from build123d import *

# Parameters (mm, degrees)
SKETCH1_W           = 20
SKETCH1_H           = 60
BOSS_EXTRUDE1_DEPTH = 15
CHAMFER1_SIZE       = 5
CUT_EXTRUDE1_DEPTH  = 36
CUT_EXTRUDE2_DEPTH  = 36
CUT_EXTRUDE3_DEPTH  = 6


with BuildPart() as part:
    # Sketch1 → Boss-Extrude1 (new body)
    with BuildSketch(Plane(origin=(0, 0, 0), x_dir=(1, 0, 0), z_dir=(0, 1, 0))):
        Rectangle(SKETCH1_W, SKETCH1_H)
    extrude(amount=BOSS_EXTRUDE1_DEPTH)

    # Chamfer1
    chamfer1_edges = [part.edges().sort_by_distance(p)[0] for p in [
        (-10, 15, 0),
    ]]
    chamfer(chamfer1_edges, length=CHAMFER1_SIZE)

    # Sketch2 → Cut-Extrude1 (cut, through all)
    with BuildSketch(Plane(origin=(0, 15, 0), x_dir=(1, 0, 0), z_dir=(0, 1, 0))):
        Polygon((10, -30), (9, -30), (10, -10), align=None)
    extrude(amount=-CUT_EXTRUDE1_DEPTH, mode=Mode.SUBTRACT)

    # Sketch3 → Cut-Extrude2 (cut, through all)
    with BuildSketch(Plane(origin=(0, 15, 0), x_dir=(1, 0, 0), z_dir=(0, 1, 0))):
        with BuildLine():
            Line((5, 21.75), (-1, 21.75))
            ThreePointArc((-1, 21.75), (-3.25, 24), (-1, 26.25))
            Line((-1, 26.25), (5, 26.25))
            ThreePointArc((5, 26.25), (7.25, 24), (5, 21.75))
        make_face()
    cut_extrude2 = extrude(amount=-CUT_EXTRUDE2_DEPTH, mode=Mode.SUBTRACT)

    # Sketch4 → Cut-Extrude3 (cut)
    with BuildSketch(Plane(origin=(0, 15, 0), x_dir=(1, 0, 0), z_dir=(0, 1, 0))):
        with BuildLine():
            Line((-1, 19.75), (5, 19.75))
            ThreePointArc((5, 19.75), (9.25, 24), (5, 28.25))
            Line((5, 28.25), (-1, 28.25))
            ThreePointArc((-1, 28.25), (-5.25, 24), (-1, 19.75))
        make_face()
    cut_extrude3 = extrude(amount=-CUT_EXTRUDE3_DEPTH, mode=Mode.SUBTRACT)

    # Mirror1: Cut-Extrude2, Cut-Extrude3 across plane
    add(cut_extrude2.mirror(Plane.XY), mode=Mode.SUBTRACT)
    add(cut_extrude3.mirror(Plane.XY), mode=Mode.SUBTRACT)


solid = part.part
Part model, mm, in its own coordinate system. A direction names the side the tool comes from. Coordinates: 2 decimals unless noted, no trailing zeros. Order: outer loops, then holes, each group sorted by start corner. A loop starts at its lowest first (then second) coordinate and runs counter-clockwise, first axis right, second up.
(1) Slice it at B-B, the plane x = 3.25. Write the cut outline in (y, z), and give its area (3 significant figures).
Check sheet entries:
outline: (0, -30) - (15, -30) - (15, -28.25) - (9, -28.25) - (9, -26.25) - (0, -26.25) - close; (0, -21.75) - (9, -21.75) - (9, -19.75) - (15, -19.75) - (15, 19.75) - (9, 19.75) - (9, 21.75) - (0, 21.75) - close; (0, 26.25) - (9, 26.25) - (9, 28.25) - (15, 28.25) - (15, 30) - (0, 30) - close
area: 717 mm2
(2) Pull direction X, two halves, no side cores. Call faces 1 (the face through (0, 7, -30)), 2 (the face through (-7, 13, 0)), 3 (the face through (2, 12, 19.75)): pulls with the +X half, pulls with the -X half, needs draft (parallel to the pull), parting line crosses it, or undercut.
Check sheet entries:
face 1: needs draft
face 2: pulls with the -X half
face 3: undercut
(3) Pin check, flat tip, straight feed: pin 1 Ø4 at (x, z) = (1, 22) entering from +Y. Stop position of the tip, or through.
Check sheet entries:
pin 1: stops at y = 9
(4) Slice it at A-A, the plane z = -24. Write the cut outline in (x, y).
Check sheet entries:
outline: (-10, 0) - (-3.25, 0) - (-3.25, 9) - (-5.25, 9) - (-5.25, 14.75) - (-10, 10) - close; (7.25, 0) - (10, 0) - (10, 15) - (9.25, 15) - (9.25, 9) - (7.25, 9) - close
(5) Slice it at C-C, the plane y = 12. Write the cut outline in (x, z), and give its area (3 significant figures).
Check sheet entries:
outline: (-8, -30) - (10, -30) - (10, 10) - (9, 30) - (-8, 30) - close; hole (-1, -28.25) - (5, -28.25) arc R4.25 ccw to (5, -19.75) - (-1, -19.75) arc R4.25 ccw to start; hole (-1, 19.75) - (5, 19.75) arc R4.25 ccw to (5, 28.25) - (-1, 28.25) arc R4.25 ccw to start
area: 855 mm2
(6) Slice it at D-D, the plane z = -13.5. Write the cut outline in (x, y).
Check sheet entries:
outline: (-10, 0) - (10, 0) - (10, 15) - (-5, 15) - (-10, 10) - close
(7) Probe L1, parallel to Z at x = 2, y = 5.5; L2, parallel to Z at x = 1.25, y = 13.5; L3, parallel to X at y = 1.25, z = -24. List the from-to ranges inside material, lowest first.
Check sheet entries:
L1: z = -30 to -26.25, -21.75 to 21.75, 26.25 to 30
L2: z = -30 to -28.25, -19.75 to 19.75, 28.25 to 30
L3: x = -10 to -3.25, 7.25 to 10
(8) Tool access for faces 4 (the face through (-1, 7, 30)), 5 (the face through (2, 12, -19.75)), 6 (the face through (2, 5, 21.75)): list every direction of +Z, -Z, +X, -X, +Y, -Y with a clear straight run to the whole face (end or side of a thin tool).
Check sheet entries:
face 4: +Z, +X, -X, +Y, -Y
face 5: +Y
face 6: +Y, -Y
